```python
from build123d import *

# Parameters (mm, degrees)
CUT_EXTRUDE1_DEPTH = 637.880050586
SKETCH3_W          = 24
SKETCH3_H          = 50


with BuildPart() as part:
    # Sketch1 → Revolve1 (revolve)
    with BuildSketch(Plane(origin=(0, 234.743963655, 0), x_dir=(1, 0, 0), z_dir=(0, 1, 0))):
        Polygon((561.230642584, 824.998443067), (521.230642584, 824.998443067), (521.230642584, 774.998443067), (563.755642584, 774.998443067), (568.730642584, 812.498443067), (568.730642584, 817.498443067), align=None)
    revolve(axis=Axis((521.230642584, 234.743963655, -824.998443067), (0, 0, 1)))

    # Sketch2 → Cut-Extrude1 (cut, through all)
    with BuildSketch(Plane.XY.offset(-774.998443067)):
        with BuildLine():
            Line((549.898349026, 234.692901362), (546.50406086, 248.275198952))
            Line((546.50406086, 248.275198952), (541.805052122, 247.10089176))
            ThreePointArc((541.805052122, 247.10089176), (544.514581311, 240.562743369), (545.199340288, 233.518594169))
            Line((545.199340288, 233.518594169), (549.898349026, 234.692901362))
        make_face()
    extrude(amount=-CUT_EXTRUDE1_DEPTH, mode=Mode.SUBTRACT)

    # Sketch3 → Cut-Revolve1 (revolve, cut)
    with BuildSketch(Plane.XZ.offset(-234.743963655)):
        with Locations((533.230642584, -799.998443067)):
            Rectangle(SKETCH3_W, SKETCH3_H)
    revolve(axis=Axis((521.230642584, 234.743963655, -774.998443067), (0, 0, -1)), mode=Mode.SUBTRACT)


solid = part.part
```
The model under review builds one solid part; all positions refer to its coordinate system, in mm. A direction names the side the tool comes from. Coordinates: 2 decimals unless noted, no trailing zeros. Write each loop counter-clockwise with the first axis right and the second up, starting at its lowest first coordinate (ties: lowest second). Pieces come first, ordered by that corner, then holes.
1) We need section A-A on z = -787. State the section outline as (x, y) points, then the cut area to 3 significant figures.
2) We need section B-B on z = -800. State the section outline as (x, y) points.
3) The part is to be moulded in two halves that separate along X. For faces 1 (the face through (503, 216, -774.998)), 2 (the face through (548.225, 241.389, -799.648)), 3 (the face through (512.5, 195.3, -824.6)), say which applies: pulls with the +X half, pulls with the -X half, needs draft (parallel to the pull), parting line crosses it, or undercut.
4) Clearance check with flat-ended pins moving along their axes: pin 1 Ø4 at (x, z) = (545.5, -818) entering from +Y; pin 2 Ø10 at (x, z) = (499, -795) entering from +Y; pin 3 Ø6 at (x, z) = (550, -787) entering from -Y; pin 4 Ø4 at (y, z) = (234, -812) entering from -X. State where each tip first meets the part, or that it passes through.
5) To check wall thickness, follow probe 1 along Y at (x, z) = (515, -808); probe 2 along X at (y, z) = (257, -812); probe 3 along Y at (x, z) = (503.5, -812). State the ranges of each line that lie inside material, in increasing order.
6) Machinability: for faces 4 (the face through (547.52, 234.1, -799.65)), 5 (the face through (545.15, 272.26, -789.84)), which of the approach directions +Z, -Z, +X, -X, +Y, -Y give a long, thin tool a straight path to every point of the face, cutting with its end or side? Answer none if there is none.
Answer list:
1. outline: circle Ø88.23 at (521.23, 234.74); hole (541.81, 247.1) arc R24 ccw (long way) to (545.2, 233.52) - (549.9, 234.69) - (546.5, 248.28) - close
1. area: 4,250 mm2
2. outline: circle Ø91.68 at (521.23, 234.74); hole (541.81, 247.1) arc R24 ccw (long way) to (545.2, 233.52) - (549.9, 234.69) - (546.5, 248.28) - close
3. face 1: needs draft
3. face 2: undercut
3. face 3: parting line crosses it
4. pin 1: stops at y = 276.67
4. pin 2: stops at y = 276.63
4. pin 3: stops at y = 198.88
4. pin 4: stops at x = 473.73
5. probe 1: y = 188.26 to 211.57, 257.92 to 281.23
5. probe 2: x = 479.34 to 512.25, 530.21 to 563.12
5. probe 3: y = 190.75 to 218.57, 250.92 to 278.74
6. face 4: +Z, -Z
6. face 5: +Z
